from build123d import *

# Parameters (mm, degrees)
BOSS_EXTRUDE1_DEPTH = 332.5
CHAMFER1_SIZE       = 15
SHELL1_T            = -2
SKETCH7_W           = 661
SKETCH7_H           = 23.794174757
CUT_EXTRUDE1_DEPTH  = 356.077808374
BOSS_EXTRUDE2_DEPTH = 665


with BuildPart() as part:
    # Sketch1 → Boss-Extrude1 (new, symmetric)
    with BuildSketch(Plane(origin=(0, 0, 0), x_dir=(0, 0, -1), z_dir=(1, 0, 0))):
        Polygon((0, 0), (40, 0), (40, -120), (14.446601942, -120), align=None)
    extrude(amount=BOSS_EXTRUDE1_DEPTH, both=True)

    # Chamfer1
    chamfer1_edges = [part.edges().sort_by_distance(p)[0] for p in [
        (0, 0, -40),
    ]]
    chamfer(chamfer1_edges, length=CHAMFER1_SIZE)

    # Shell1
    shell1_openings = [part.faces().sort_by_distance(p)[0] for p in [
        (0, -60, -7.223300971),
    ]]
    offset(amount=SHELL1_T, openings=shell1_openings, kind=Kind.INTERSECTION)

    # Sketch7 → Cut-Extrude1 (cut, through all)
    with BuildSketch(Plane(origin=(0, -118, 0), x_dir=(1, 0, 0), z_dir=(0, 1, 0))):
        with Locations((0, 26.102912621)):
            Rectangle(SKETCH7_W, SKETCH7_H)
    extrude(amount=-CUT_EXTRUDE1_DEPTH, mode=Mode.SUBTRACT)

    # Sketch8 → Boss-Extrude2 (add)
    with BuildSketch(Plane(origin=(332.5, 0, 0), x_dir=(0, 0, -1), z_dir=(1, 0, 0))):
        with BuildLine():
            Line((40, -120), (55.171572875, -120))
            ThreePointArc((55.171572875, -120), (55.93693974, -119.847759065), (56.585786438, -119.414213562))
            Line((56.585786438, -119.414213562), (68.02081528, -107.97918472))
            Line((68.02081528, -107.97918472), (66.606601718, -106.564971157))
            Line((66.606601718, -106.564971157), (55.757359313, -117.414213562))
            ThreePointArc((55.757359313, -117.414213562), (55.108512615, -117.847759065), (54.343145751, -118))
            Line((54.343145751, -118), (40, -118))
            Line((40, -118), (40, -120))
        make_face()
    extrude(amount=-BOSS_EXTRUDE2_DEPTH)


solid = part.part
Read the model definition and answer for the solid it produces. Units are mm, in the model's axes. A direction names the side the tool comes from. Give positions to 0.01 mm unless a question says otherwise; leave off trailing zeros. Write each loop counter-clockwise with the first axis right and the second up, starting at its lowest first coordinate (ties: lowest second). Pieces come first, ordered by that corner, then holes. Notation, with made-up numbers: (78.5, 76.25) - (99.5, 76.25) arc R13 ccw to (99.5, 88.25) - close; hole circle Ø10 at (0, 88). An arc over 180 degrees is marked (long way). Answer in a Markdown table with one row per item. Add a question column.
Item 1: Determine the mould class of faces 1 (the face through (5, -114, -62)), 2 (the face through (-332.5, -59, -18)), 3 (the face through (-5, -67, -38)) for opening direction X: pulls with the +X half, pulls with the -X half, needs draft (parallel to the pull), parting line crosses it, or undercut.
Item 2: Section B-B, the plane x = -189 is taken. Write down the section's boundary in (y, z).
Item 3: Section C-C, the plane z = -6.5 is taken. Write down the section's boundary in (x, y), and give its area (3 significant figures).
Item 4: Flat-ended cylindrical pins translate along their axes: P1, Ø8, axis at x = 158, z = -31, coming from the -Y side; P2, Ø2, axis at x = -165, y = -83, coming from the +Z side; P3, Ø7, axis at x = 6.5, z = -49.5, coming from the +Y side. Find the tip coordinate at first contact, or state that the pin passes through.
Item 5: Section A-A, the plane y = -76 is taken. Write down the section's boundary in (x, z), and give its area (3 significant figures).
Item 6: Find the intervals of material crossed by L1, parallel to X at y = -87.5, z = -35.5; L2, parallel to Y at x = 103.5, z = -6.5; L3, parallel to Z at x = -174, y = -51, in increasing order.
Item 7: A tool of negligible diameter and unlimited length cuts with its end or side. For faces 4 (the face through (-330.5, -60, -23)), 5 (the face through (332.5, -59, -18)), 6 (the face through (5, -118, -47)), from which of +Z, -Z, +X, -X, +Y, -Y can it reach the whole face along a straight path? Write none if from no direction.
Item 8: Section D-D, the plane z = -47.5 is taken. Write down the section's boundary in (x, y).
Recorded:
| question | item | result |
|---|---|---|
| 1 | face 1 | needs draft |
| 1 | face 2 | pulls with the -X half |
| 1 | face 3 | undercut |
| 2 | outline | (-120, -55.17) arc R2 ccw to (-119.41, -56.59) - (-107.98, -68.02) - (-106.56, -66.61) - (-117.41, -55.76) arc R2 cw to (-118, -54.34) - (-118, -40) - (-15, -40) - (0, -25) - (0, 0) - (-2, -0.24) - (-2, -24.17) - (-15.83, -38) - (-120, -38) - close |
| 3 | outline | (-332.5, -53.99) - (-330.5, -53.99) - (-330.5, -2) - (330.5, -2) - (330.5, -53.99) - (332.5, -53.99) - (332.5, 0) - (-332.5, 0) - close |
| 3 | area | 1,540 mm2 |
| 4 | P1 | stops at y = -12.83 |
| 4 | P2 | stops at z = -38 |
| 4 | P3 | stops at y = -118 |
| 5 | outline | (-332.5, -40) - (332.5, -40) - (332.5, -9.15) - (330.5, -9.15) - (330.5, -38) - (-330.5, -38) - (-330.5, -9.15) - (-332.5, -9.15) - close |
| 5 | area | 1,450 mm2 |
| 6 | L1 | x = -332.5 to -330.5, 330.5 to 332.5 |
| 6 | L2 | y = -2 to 0 |
| 6 | L3 | z = -40 to -38 |
| 7 | face 4 | +Z, -Y |
| 7 | face 5 | +Z, -Z, +X, +Y, -Y |
| 7 | face 6 | +X, -X, +Y |
| 8 | outline | (-332.5, -120) - (332.5, -120) - (332.5, -118) - (-332.5, -118) - close |
